from build123d import *

# Parameters (mm, degrees)
SKETCH1_W           = 33
SKETCH1_H           = 60
SKETCH1_R           = 2.25
SKETCH1_R_2         = 1.75
BOSS_EXTRUDE1_DEPTH = 2
CHAMFER1_SIZE       = 2


with BuildPart() as part:
    # Sketch1 → Boss-Extrude1 (new body)
    with BuildSketch(Plane.XY):
        Rectangle(SKETCH1_W, SKETCH1_H)
        with Locations((0, 7)):
            Circle(SKETCH1_R, mode=Mode.SUBTRACT)
        with Locations((13.5, -26)):
            Circle(SKETCH1_R_2, mode=Mode.SUBTRACT)
        with Locations((-13.5, -8)):
            Circle(SKETCH1_R_2, mode=Mode.SUBTRACT)
        with BuildLine():
            ThreePointArc((9.01561146, 16.01561146), (0, 19.75), (-9.01561146, 16.01561146))
            ThreePointArc((-9.01561146, 16.01561146), (-12.197591975, 16.01561146), (-12.197591975, 19.197591975))
            ThreePointArc((-12.197591975, 19.197591975), (0, 24.25), (12.197591975, 19.197591975))
            ThreePointArc((12.197591975, 19.197591975), (12.197591975, 16.01561146), (9.01561146, 16.01561146))
        make_face(mode=Mode.SUBTRACT)
    extrude(amount=BOSS_EXTRUDE1_DEPTH)

    # Chamfer1
    chamfer1_edges = [part.edges().sort_by_distance(p)[0] for p in [
        (16.5, -30, 1),
        (-16.5, -30, 1),
        (-16.5, 30, 1),
        (16.5, 30, 1),
    ]]
    chamfer(chamfer1_edges, length=CHAMFER1_SIZE)


solid = part.part
The model under review builds one solid part; all positions refer to its coordinate system, in mm. A direction names the side the tool comes from. Coordinates: 2 decimals unless noted, no trailing zeros. Write each loop counter-clockwise with the first axis right and the second up, starting at its lowest first coordinate (ties: lowest second). Pieces come first, ordered by that corner, then holes. Notation, with made-up numbers: M 20.5,-9 L 75.5,-9 A18 ccw 75.5,15 Z; hole C 78.5,34 d7. An arc over 180 degrees is marked long. Put each result on its own line as item: value.
1) Add section C-C on z = 0.9. Give the boundary of the cut face in (x, y).
Computed:
outline: M -16.5,-28 L -14.5,-30 L 14.5,-30 L 16.5,-28 L 16.5,28 L 14.5,30 L -14.5,30 L -16.5,28 Z; hole C -13.5,-8 d3.5; hole M -12.2,19.2 A2.25 ccw -9.02,16.02 A12.75 cw 9.02,16.02 A2.25 ccw 12.2,19.2 A17.25 ccw Z; hole C 0,7 d4.5; hole C 13.5,-26 d3.5
2) Wall thickness on probe 1 along Y at (x, z) = (0, 0.8); probe 2 along Y at (x, z) = (13.5, 1.45); probe 3 along Y at (x, z) = (-13.5, 0.65): over which ranges is each line inside the solid? List them lowest first. Write a range as [from, to].
Computed:
probe 1: y = [-30, 4.75], [9.25, 19.75], [24.25, 30]
probe 2: y = [-30, -27.75], [-24.25, 30]
probe 3: y = [-30, -9.75], [-6.25, 30]
3) Draft analysis for pull direction Y (two halves, no side actions). For faces 1 (the cylindrical face through (-0.19, 24.25, 0.99)), 2 (the flat face through (-15.5, -29, 1)), 3 (the flat face through (0, 0, 2)), state which applies: released by +Y, released by -Y, zero draft, split by the parting line, or undercut.
Computed:
face 1: undercut
face 2: released by -Y
face 3: zero draft
4) For faces 4 (the flat face through (0, 30, 1)), 5 (the cylindrical face through (0.14, 19.75, 0.99)), list the 3-axis set-ups (+Z, -Z, +X, -X, +Y, -Y) from which the entire face can be reached by the end or side of a thin tool; tool diameter is ignored.
Computed:
face 4: +Z, -Z, +X, -X, +Y
face 5: +Z, -Z
5) Add section D-D on x = -13.5. Give the boundary of the cut face in (y, z).
Computed:
outline: M -30,0 L -9.75,0 L -9.75,2 L -30,2 Z; M -6.25,0 L 30,0 L 30,2 L -6.25,2 Z
6) Add section A-A on y = -8. Give the boundary of the cut face in (x, z).
Computed:
outline: M -16.5,0 L -15.25,0 L -15.25,2 L -16.5,2 Z; M -11.75,0 L 16.5,0 L 16.5,2 L -11.75,2 Z
7) Add section B-B on x = 0. Give the boundary of the cut face in (y, z).
Computed:
outline: M -30,0 L 4.75,0 L 4.75,2 L -30,2 Z; M 9.25,0 L 19.75,0 L 19.75,2 L 9.25,2 Z; M 24.25,0 L 30,0 L 30,2 L 24.25,2 Z
